```python
from build123d import *

# Parameters (mm, degrees)
SKETCH_1_W          = 90
SKETCH_1_H          = 250
EXTRUDE_1_DEPTH     = 5
SKETCH_2_R          = 2.5
SKETCH_2_R_2        = 2.1
CUT_EXTRUDE_1_DEPTH = 5
SKETCH_3_R          = 2.75
CUT_EXTRUDE_2_DEPTH = 5
SKETCH_4_R          = 2.75
CUT_EXTRUDE_3_DEPTH = 5
FILLET_1_R          = 5


with BuildPart() as part:
    # 草图1 → 凸台-拉伸1 (new body)
    with BuildSketch(Plane.XY):
        Rectangle(SKETCH_1_W, SKETCH_1_H)
    extrude(amount=EXTRUDE_1_DEPTH)

    # 草图2 → 切除-拉伸1 (cut)
    with BuildSketch(Plane.XY.offset(5)):
        with Locations((0, 110)):
            Circle(SKETCH_2_R)
        with Locations((0, 85)):
            Circle(SKETCH_2_R)
        with Locations((-30, 42)):
            Circle(SKETCH_2_R_2)
        with Locations((30, 42)):
            Circle(SKETCH_2_R_2)
    extrude(amount=-CUT_EXTRUDE_1_DEPTH, mode=Mode.SUBTRACT)

    # 草图3 → 切除-拉伸2 (cut)
    with BuildSketch(Plane.XY.offset(5)):
        with Locations((-20, -30)):
            Circle(SKETCH_3_R)
        with Locations((20, -30)):
            Circle(SKETCH_3_R)
        with Locations((0, -80)):
            Circle(SKETCH_3_R)
        with Locations((0, -70)):
            Circle(SKETCH_3_R)
        with Locations((0, -60)):
            Circle(SKETCH_3_R)
        with Locations((0, -50)):
            Circle(SKETCH_3_R)
        with Locations((0, -40)):
            Circle(SKETCH_3_R)
        with Locations((0, -90)):
            Circle(SKETCH_3_R)
        with Locations((0, -100)):
            Circle(SKETCH_3_R)
        with Locations((0, -110)):
            Circle(SKETCH_3_R)
        with Locations((-20, -20)):
            Circle(SKETCH_3_R)
        with Locations((20, -20)):
            Circle(SKETCH_3_R)
        with Locations((-20, -10)):
            Circle(SKETCH_3_R)
        with Locations((20, -10)):
            Circle(SKETCH_3_R)
        with Locations((-20, 0)):
            Circle(SKETCH_3_R)
        with Locations((20, 0)):
            Circle(SKETCH_3_R)
        with Locations((-20, 10)):
            Circle(SKETCH_3_R)
        with Locations((20, 10)):
            Circle(SKETCH_3_R)
    extrude(amount=-CUT_EXTRUDE_2_DEPTH, mode=Mode.SUBTRACT)

    # 草图4 → 切除-拉伸3 (cut)
    with BuildSketch(Plane.XY.offset(5)):
        with Locations((-30, -113)):
            Circle(SKETCH_4_R)
        with Locations((30, -113)):
            Circle(SKETCH_4_R)
        with Locations((-30, -103)):
            Circle(SKETCH_4_R)
        with Locations((30, -103)):
            Circle(SKETCH_4_R)
        with Locations((-30, -93)):
            Circle(SKETCH_4_R)
        with Locations((30, -93)):
            Circle(SKETCH_4_R)
        with Locations((-30, -83)):
            Circle(SKETCH_4_R)
        with Locations((30, -83)):
            Circle(SKETCH_4_R)
        with Locations((-30, -73)):
            Circle(SKETCH_4_R)
        with Locations((30, -73)):
            Circle(SKETCH_4_R)
    extrude(amount=-CUT_EXTRUDE_3_DEPTH, mode=Mode.SUBTRACT)

    # 圆角1
    fillet_1_edges = [part.edges().sort_by_distance(p)[0] for p in [
        (45, -125, 2.5),
        (-45, -125, 2.5),
        (-45, 125, 2.5),
        (45, 125, 2.5),
    ]]
    fillet(fillet_1_edges, radius=FILLET_1_R)


solid = part.part
```
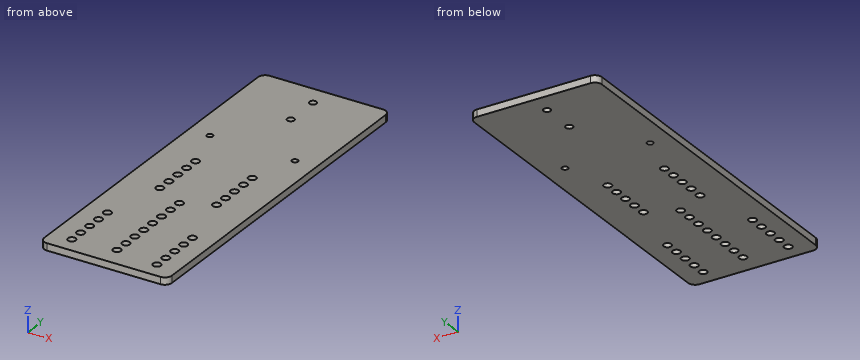
Read the model definition and answer for the solid it produces. Units are mm, in the model's axes. Coordinates: 2 decimals unless noted, no trailing zeros. Write each loop counter-clockwise with the first axis right and the second up, starting at its lowest first coordinate (ties: lowest second). Pieces come first, ordered by that corner, then holes. Notation, with made-up numbers: (-0.75, 34.5) -> (8.25, 34.5) arc R30 cw to (8.25, 61.5) -> close; hole circle Ø11 at (36.5, -27). An arc over 180 degrees is marked (long way). Answer as a JSON object with one key per item and string values.
Q1. Consider line 1 (Y direction, x = -20, z = 1.55); line 2 (Y direction, x = -22.5, z = 3); line 3 (X direction, y = 83, z = 2.4). Determine where each line is inside the solid, lowest interval first. Write a range as [from, to].
The answers:
{"line 1": "y = [-125, -32.75], [-27.25, -22.75], [-17.25, -12.75], [-7.25, -2.75], [2.75, 7.25], [12.75, 125]", "line 2": "y = [-125, -31.15], [-28.85, -21.15], [-18.85, -11.15], [-8.85, -1.15], [1.15, 8.85], [11.15, 125]", "line 3": "x = [-45, -1.5], [1.5, 45]"}
Q2. The part is cut by section A-A on y = -50. Give the vertices of the cut face in (x, z).
The answers:
{"outline": "(-45, 0) -> (-2.75, 0) -> (-2.75, 5) -> (-45, 5) -> close; (2.75, 0) -> (45, 0) -> (45, 5) -> (2.75, 5) -> close"}
Q3. The part is cut by section C-C on z = 2.9. Give the number of separate pieces and of enclosed holes in the cut face, then the cut area to 3 significant figures.
The answers:
{"separate pieces": "1", "enclosed holes": "32", "area": "21,700 mm2"}
Q4. The part is cut by section B-B on y = -10. Give the vertices of the cut face in (x, z), then the cut area to 3 significant figures.
The answers:
{"outline": "(-45, 0) -> (-22.75, 0) -> (-22.75, 5) -> (-45, 5) -> close; (-17.25, 0) -> (17.25, 0) -> (17.25, 5) -> (-17.25, 5) -> close; (22.75, 0) -> (45, 0) -> (45, 5) -> (22.75, 5) -> close", "area": "395 mm2"}
